Could you check a few things on this model? Use its own coordinates, in mm. Give positions to 0.01 mm unless a question says otherwise; leave off trailing zeros. Loops run counter-clockwise (first coordinate to the right, second up) from the corner with the lowest first, then second, coordinate; pieces in that order, holes last. Notation, with made-up numbers: (59.25, -16.5) - (93.25, -16.5) arc R22 cw to (93.25, 11.5) - close; hole circle Ø5 at (-14.75, 30.5). An arc over 180 degrees is marked (long way). Use CSV: the item, a comma, the result in double quotes.
from build123d import *

# Parameters (mm, degrees)
SKETCH_1_W                   = 200
SKETCH_1_H                   = 330
EXTRUDE_1_DEPTH              = 7.5
HOLE_WIZARD_M6_1_D           = 6.6
HOLE_WIZARD_M6_1_CBORE_D     = 11
HOLE_WIZARD_M6_1_CBORE_DEPTH = 8
HOLE_WIZARD_M6_2_D           = 6.6
HOLE_WIZARD_M6_2_CBORE_D     = 11
HOLE_WIZARD_M6_2_CBORE_DEPTH = 8
HOLE_WIZARD_M6_1_2_D         = 5
HOLE_WIZARD_M6_1_2_DEPTH     = 17
HOLE_WIZARD_M6_1_2_TIP       = 1.502151548


with BuildPart() as part:
    # 草图1 → 凸台-拉伸1 (new, symmetric)
    with BuildSketch(Plane(origin=(0, 0, 0), x_dir=(1, 0, 0), z_dir=(0, 1, 0))):
        Rectangle(SKETCH_1_W, SKETCH_1_H)
    extrude(amount=EXTRUDE_1_DEPTH, both=True)

    # Hole Wizard M6 _1 (through all)
    with Locations(Plane(origin=(0, -7.5, 0), x_dir=(-1, 0, 0), z_dir=(0, -1, 0))):
        with Locations((0, 0), (0, -125), (0, 125)):
            CounterBoreHole(HOLE_WIZARD_M6_1_D / 2, HOLE_WIZARD_M6_1_CBORE_D / 2, HOLE_WIZARD_M6_1_CBORE_DEPTH)

    # M6 六角凹头螺钉的柱形沉头孔2 (through all)
    with Locations(Plane(origin=(0, -7.5, 0), x_dir=(-1, 0, 0), z_dir=(0, -1, 0))):
        with Locations((85, 155), (0, 155), (-85, 155)):
            CounterBoreHole(HOLE_WIZARD_M6_2_D / 2, HOLE_WIZARD_M6_2_CBORE_D / 2, HOLE_WIZARD_M6_2_CBORE_DEPTH)

    # Hole Wizard M6 _1 2
    with Locations(Plane.XY.offset(165)):
        with Locations((0, 0), (-90, 0), (90, 0)):
            Hole(HOLE_WIZARD_M6_1_2_D / 2, depth=HOLE_WIZARD_M6_1_2_DEPTH)
            with Locations((0, 0, -(HOLE_WIZARD_M6_1_2_DEPTH + HOLE_WIZARD_M6_1_2_TIP / 2))):  # 118° drill point
                Cone(0, HOLE_WIZARD_M6_1_2_D / 2, HOLE_WIZARD_M6_1_2_TIP, mode=Mode.SUBTRACT)


solid = part.part
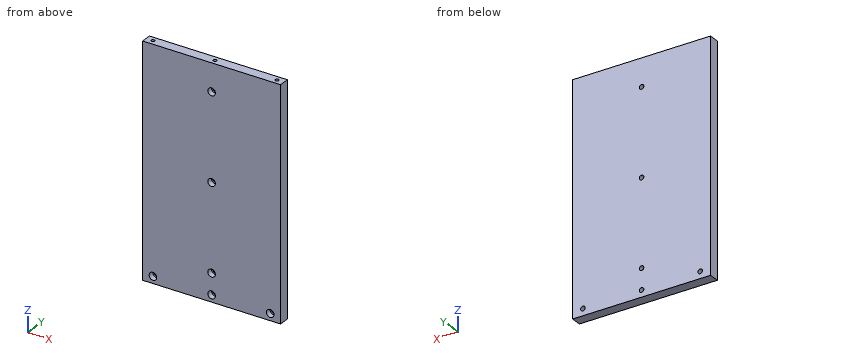
1) I need wall thicknesses on line 1 along X through (y, z) = (0, 159.5); line 2 along Z through (x, y) = (0, -4); line 3 along Z through (x, y) = (0, 4). Which ranges of each line are inside material? Lowest first, please.
Answer below:
line 1,"x = -100 to -92.5, -87.5 to -2.5, 2.5 to 87.5, 92.5 to 100"
line 2,"z = -165 to -160.5, -149.5 to -130.5, -119.5 to -5.5, 5.5 to 119.5, 130.5 to 165"
line 3,"z = -165 to -158.3, -151.7 to -128.3, -121.7 to -3.3, 3.3 to 121.7, 128.3 to 165"
2) I'm going to push a flat-ended pin straight in: P1, Ø5.5, axis at x = 2, z = 126, coming from the -Y side. Where does the tip first touch, or does it pass through?
Answer below:
P1,"stops at y = 0.5"
3) Suppose I cut it at B-B (z = -155). Please give me the cut outline in (x, y).
Answer below:
outline,"(-100, -7.5) - (-90.5, -7.5) - (-90.5, 0.5) - (-88.3, 0.5) - (-88.3, 7.5) - (-100, 7.5) - close; (-81.7, 0.5) - (-79.5, 0.5) - (-79.5, -7.5) - (-5.5, -7.5) - (-5.5, 0.5) - (-3.3, 0.5) - (-3.3, 7.5) - (-81.7, 7.5) - close; (3.3, 0.5) - (5.5, 0.5) - (5.5, -7.5) - (79.5, -7.5) - (79.5, 0.5) - (81.7, 0.5) - (81.7, 7.5) - (3.3, 7.5) - close; (88.3, 0.5) - (90.5, 0.5) - (90.5, -7.5) - (100, -7.5) - (100, 7.5) - (88.3, 7.5) - close"
4) Suppose I cut it at A-A (z = 0). Please give me the cut outline in (x, y), plus the area to 3 significant figures.
Answer below:
outline,"(-100, -7.5) - (-5.5, -7.5) - (-5.5, 0.5) - (-3.3, 0.5) - (-3.3, 7.5) - (-100, 7.5) - close; (3.3, 0.5) - (5.5, 0.5) - (5.5, -7.5) - (100, -7.5) - (100, 7.5) - (3.3, 7.5) - close"
area,"2,870 mm2"
